Geometry check sheet. Reference: drawing and pictorial views, mm from the part's lowest x, y, z. A direction names the side the tool comes from. Coordinates: 2 decimals unless noted, no trailing zeros. Loops run counter-clockwise (first coordinate to the right, second up) from the corner with the lowest first, then second, coordinate; pieces in that order, holes last. Notation, with made-up numbers: (0, 86) -> (39, 86) arc R24 ccw to (39, 98) -> close; hole circle Ø9 at (46, 49). An arc over 180 degrees is marked (long way). Answer as a JSON object with one key per item and string values. Group by question number.
Q1. Gauge pin test, flat ends, axial feed: pin 1 Ø1 at (y, z) = (2.5, 2) entering from +X; pin 2 Ø5 at (x, y) = (9.5, 3) entering from -Z. Record the tip position at first contact, or that the pin passes through.
Q2. Set-up check for the marked faces 1, 2 and 3: record each of +Z, -Z, +X, -X, +Y, -Y from which the full face is reachable in a straight line by a thin tool's end or side.
Q3. Cross-section at A-A on z = 1.6. Record the boundary of the cut face in (x, y), and give its area (3 significant figures).
Q4. Cross-section at B-B on y = 21.5. Record the boundary of the cut face in (x, z), and give its area (3 significant figures).
Q5. Scan lines: L1, parallel to X at y = 2, z = 3; L2, parallel to Y at x = 2.5, z = 0.45. Record each from-to range of solid material in increasing order.
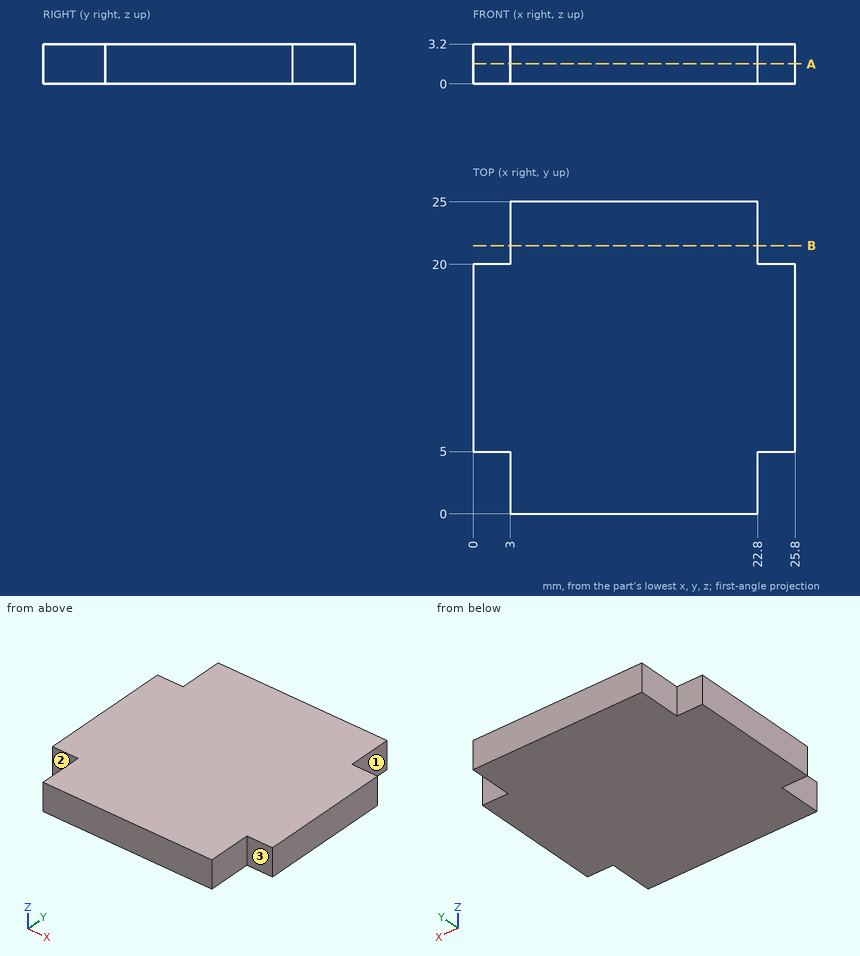
Computed values:
{
 "1": {"pin 1": "stops at x = 22.8", "pin 2": "stops at z = 0"},
 "2": {"face 1": "+Z, -Z, +X, +Y", "face 2": "+Z, -Z, -X, -Y", "face 3": "+Z, -Z, +X, -Y"},
 "3": {"outline": "(0, 5) -> (3, 5) -> (3, 0) -> (22.8, 0) -> (22.8, 5) -> (25.8, 5) -> (25.8, 20) -> (22.8, 20) -> (22.8, 25) -> (3, 25) -> (3, 20) -> (0, 20) -> close", "area": "585 mm²"},
 "4": {"outline": "(3, 0) -> (22.8, 0) -> (22.8, 3.2) -> (3, 3.2) -> close", "area": "63.4 mm²"},
 "5": {"L1": "x = 3 to 22.8", "L2": "y = 5 to 20"}
}
